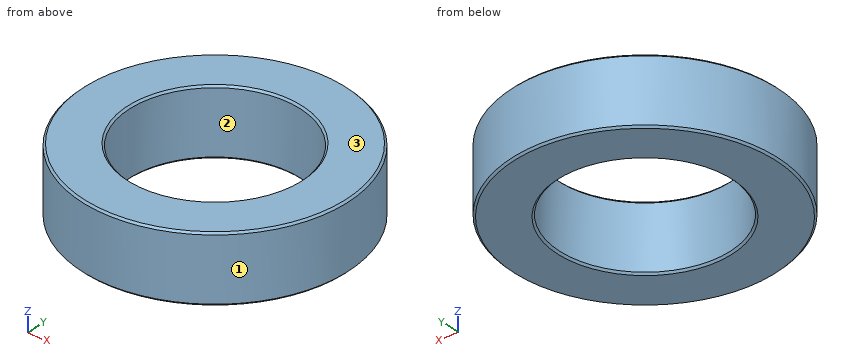
```python
from build123d import *

# Parameters (mm, degrees)
SKETCH_1_R      = 35
SKETCH_1_R_2    = 22.5
EXTRUDE_1_DEPTH = 17.5
CHAMFER_1_SIZE  = 0.5


with BuildPart() as part:
    # 草图1 → 凸台-拉伸1 (new body)
    with BuildSketch(Plane.XY):
        Circle(SKETCH_1_R)
        Circle(SKETCH_1_R_2, mode=Mode.SUBTRACT)
    extrude(amount=EXTRUDE_1_DEPTH)

    # 倒角1
    chamfer_1_edges = [part.edges().sort_by_distance(p)[0] for p in [
        (-35, 0, 0),
        (-35, 0, 17.5),
        (-22.5, 0, 0),
        (-22.5, 0, 17.5),
    ]]
    chamfer(chamfer_1_edges, length=CHAMFER_1_SIZE)


solid = part.part
```
Read the model definition and answer for the solid it produces. Units are mm, in the model's axes. Face numbers are marked on the shaded views. Round coordinates to 2 decimals unless told otherwise and drop trailing zeros. Write each loop counter-clockwise with the first axis right and the second up, starting at its lowest first coordinate (ties: lowest second). Pieces come first, ordered by that corner, then holes. Notation, with made-up numbers: M 27.5,22.5 L 83.5,22.5 A25 cw 83.5,48.5 Z; hole C 57.5,-23 d5. An arc over 180 degrees is marked long. One line per item, written item: value.
Q1. Straight lines are drawn through the part: line 1 (Y direction, x = 0, z = 8.5); line 2 (Y direction, x = -15, z = 12); line 3 (X direction, y = -18, z = 11.5). For each, find the intervals that lie inside material, in ascending order. Write a range as [from, to].
Data:
line 1: [-35, -22.5], [22.5, 35]
line 2: [-31.62, -16.77], [16.77, 31.62]
line 3: [-30.02, -13.5], [13.5, 30.02]
Q2. Find section C-C on z = 11. Write down the section's boundary in (x, y), plus the area to 3 significant figures.
Data:
outline: C 0,0 d70; hole C 0,0 d45
area: 2,260 mm2
Q3. Flat-ended cylindrical pins translate along their axes: pin 1 Ø8 at (x, z) = (18.5, 14) entering from +Y; pin 2 Ø5 at (y, z) = (12.5, 12) entering from +X; pin 3 Ø1 at (x, z) = (-3, 4) entering from +Y; pin 4 Ø2 at (x, y) = (14.5, 15.5) entering from -Z. Find the tip coordinate at first contact, or state that the pin passes through.
Data:
pin 1: y = 31.86
pin 2: x = 33.54
pin 3: y = 34.91
pin 4: through
Q4. For a pull along X with two mould halves and no side action, classify the marked faces 1, 2 and 3 as +X half, -X half, draft (parallel to the pull), parting line (faces both ways), or undercut.
Data:
face 1: parting line
face 2: undercut
face 3: draft
Q5. Find section A-A on x = 0. Write down the section's boundary in (y, z), plus the area to 4 significant figures.
Data:
outline: M -35,0.5 L -34.5,0 L -23,0 L -22.5,0.5 L -22.5,17 L -23,17.5 L -34.5,17.5 L -35,17 Z; M 22.5,0.5 L 23,0 L 34.5,0 L 35,0.5 L 35,17 L 34.5,17.5 L 23,17.5 L 22.5,17 Z
area: 436.5 mm2
